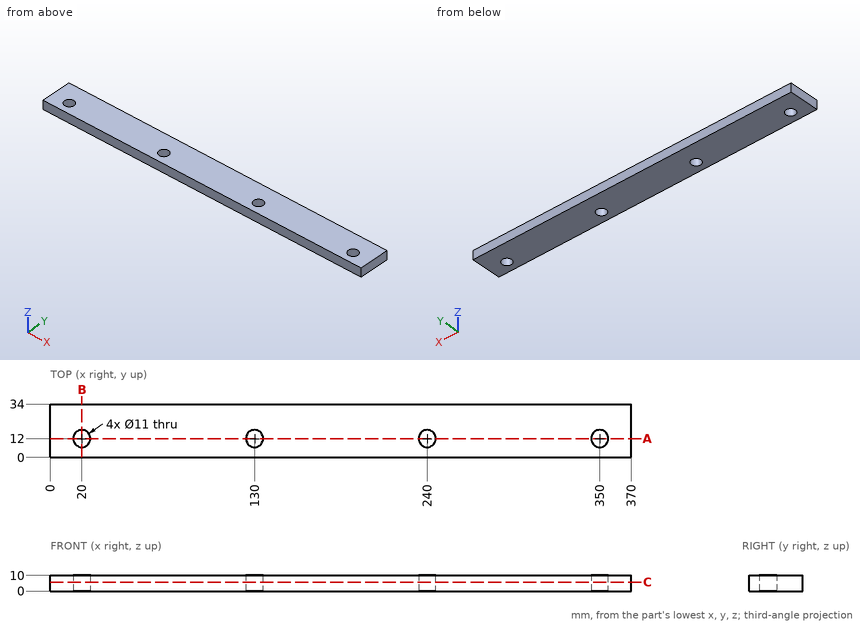
The figure shows three views and two pictorial views of one solid part (mm, origin at its lowest corner). Answer the questions. Give positions to 0.01 mm unless a question says otherwise; leave off trailing zeros. Order: outer loops, then holes, each group sorted by start corner. A loop starts at its lowest first (then second) coordinate and runs counter-clockwise, first axis right, second up. Notation, with made-up numbers: (77, 88.25) -> (119, 88.25) arc R34 cw to (119, 118.25) -> close; hole circle Ø10 at (-4.5, -36.5). An arc over 180 degrees is marked (long way). Answer as CSV lines item,"result". Start each with the question number.
Q1. Find the intervals of material crossed by L1, parallel to Y at x = 350, z = 2; L2, parallel to X at y = 10, z = 6.5; L3, parallel to X at y = 11.5, z = 4.75, in increasing order.
Q2. A cutting plane is placed at B-B (x = 20). Determine the outline of the cut face in (y, z).
Q3. A cutting plane is placed at C-C (z = 5.75). Determine the outline of the cut face in (x, y), then the cut area to 3 significant figures.
Q4. A cutting plane is placed at A-A (y = 12). Determine the outline of the cut face in (x, z), then the cut area to 3 significant figures.
Results found:
1,L1,"0 to 6.5, 17.5 to 34"
1,L2,"0 to 14.88, 25.12 to 124.88, 135.12 to 234.88, 245.12 to 344.88, 355.12 to 370"
1,L3,"0 to 14.52, 25.48 to 124.52, 135.48 to 234.52, 245.48 to 344.52, 355.48 to 370"
2,outline,"(0, 0) -> (6.5, 0) -> (6.5, 10) -> (0, 10) -> close; (17.5, 0) -> (34, 0) -> (34, 10) -> (17.5, 10) -> close"
3,outline,"(0, 0) -> (370, 0) -> (370, 34) -> (0, 34) -> close; hole circle Ø11 at (20, 12); hole circle Ø11 at (130, 12); hole circle Ø11 at (240, 12); hole circle Ø11 at (350, 12)"
3,area,"12,200 mm2"
4,outline,"(0, 0) -> (14.5, 0) -> (14.5, 10) -> (0, 10) -> close; (25.5, 0) -> (124.5, 0) -> (124.5, 10) -> (25.5, 10) -> close; (135.5, 0) -> (234.5, 0) -> (234.5, 10) -> (135.5, 10) -> close; (245.5, 0) -> (344.5, 0) -> (344.5, 10) -> (245.5, 10) -> close; (355.5, 0) -> (370, 0) -> (370, 10) -> (355.5, 10) -> close"
4,area,"3,260 mm2"
